Build history of the part. All positions in model axes, mm. A direction names the side the tool comes from. Give positions to 0.01 mm unless a question says otherwise; leave off trailing zeros. Write each loop counter-clockwise with the first axis right and the second up, starting at its lowest first coordinate (ties: lowest second). Pieces come first, ordered by that corner, then holes. Notation, with made-up numbers: M -34.5,-17.75 L -2.5,-17.75 A26 cw -2.5,4.25 Z; hole C -5.75,8 d10. An arc over 180 degrees is marked long. Return JSON: item names as keys, results as strings. Group by question number.
Q1. Wall check: probe 1 along Y at (x, z) = (-55, 27); probe 2 along Y at (x, z) = (-36.71, 14.75) (3 decimals); probe 3 along Y at (x, z) = (-51, 4). Give the ranges that are in metal, low to high.
Q2. Flat gauge pins, fed straight in: pin 1 Ø16 at (x, y) = (-55, 55) entering from -Z; pin 2 Ø10 at (x, y) = (36.71, -52.425) entering from +Z; pin 3 Ø9.5 at (x, y) = (53, -59.5) entering from -Z. Where does each tip first touch, or does it go through?
Q3. Tool access for faces 1 (the cylindrical face through (-48.371, 37.987, 12.422)), 2 (the cylindrical face through (16.128, -25.296, 33.997)): list every direction of +Z, -Z, +X, -X, +Y, -Y with a clear straight run to the whole face (end or side of a thin tool).
Q4. Pull direction Y, two halves, no side cores. Call faces 3 (the cylindrical face through (45.939, 57.854, 19.72)), 4 (the flat face through (-1, -67, 33)), 5 (the flat face through (-60, 1, 67)): +Y half, -Y half, draft (parallel to the pull), parting line (faces both ways), or undercut.
Q5. Band-saw the part on C-C, the plane z = 54. Give the cut face in (x, y), then the cut area to 3 significant figures.
Q6. Band-saw the part on A-A, the plane y = 0. Give the cut face in (x, z), then the cut area to 3 significant figures.
Q7. Band-saw the part on D-D, the plane z = 21.5. Count the separate pieces of the cut face and the enclosed holes in it, then the cut area to 3 significant figures.
from build123d import *

# Parameters (mm, degrees)
SKETCH1_W                  = 134
SKETCH1_H                  = 134
BOSS_EXTRUDE1_DEPTH        = 67
FILLET1_R                  = 12
SKETCH2_R                  = 30
CUT_EXTRUDE1_DEPTH         = 67
BOSS_EXTRUDE2_START        = 2
SKETCH3_R                  = 58
SKETCH3_R_2                = 30
BOSS_EXTRUDE2_DEPTH        = 2
SKETCH4_R                  = 58
SKETCH4_R_2                = 30
BOSS_EXTRUDE3_DEPTH        = 2
SKETCH5_R                  = 7
CUT_EXTRUDE2_DEPTH         = 160
SKETCH6_R                  = 9.5
CUT_EXTRUDE3_DEPTH         = 40
SIZE_MM_DOWEL_HOLE_1_D     = 8.5
SIZE_MM_DOWEL_HOLE_1_DEPTH = 24.5
SIZE_MM_DOWEL_HOLE_1_TIP   = 2.553657631
SIZE_MM_DOWEL_HOLE_2_D     = 8.5
SIZE_MM_DOWEL_HOLE_2_DEPTH = 24.5
SIZE_MM_DOWEL_HOLE_2_TIP   = 2.553657631
SIZE_MM_DOWEL_HOLE_3_D     = 8.6
SIZE_MM_DOWEL_HOLE_3_DEPTH = 10
SIZE_MM_DOWEL_HOLE_3_TIP   = 2.583700662


with BuildPart() as part:
    # Sketch1 → Boss-Extrude1 (new body)
    with BuildSketch(Plane.XY):
        Rectangle(SKETCH1_W, SKETCH1_H)
    extrude(amount=BOSS_EXTRUDE1_DEPTH)

    # Fillet1
    fillet1_edges = [part.edges().sort_by_distance(p)[0] for p in [
        (-67, 67, 33.5),
        (67, 67, 33.5),
        (67, -67, 33.5),
        (-67, -67, 33.5),
    ]]
    fillet(fillet1_edges, radius=FILLET1_R)

    # Sketch2 → Cut-Extrude1 (cut)
    with BuildSketch(Plane.XY.offset(67)):
        Circle(SKETCH2_R)
    extrude(amount=-CUT_EXTRUDE1_DEPTH, mode=Mode.SUBTRACT)

    # Sketch3 → Boss-Extrude2 (add)
    with BuildSketch(Plane.XY.offset(67).offset(BOSS_EXTRUDE2_START)):
        Circle(SKETCH3_R)
        Circle(SKETCH3_R_2, mode=Mode.SUBTRACT)
    extrude(amount=-BOSS_EXTRUDE2_DEPTH)

    # Sketch4 → Boss-Extrude3 (add)
    with BuildSketch(Plane(origin=(0, 0, 0), x_dir=(-1, 0, 0), z_dir=(0, 0, -1))):
        with Locations(Location((0, 0, 0), (0, 0, 180))):
            Circle(SKETCH4_R)
        with Locations(Location((0, 0, 0), (0, 0, 180))):
            Circle(SKETCH4_R_2, mode=Mode.SUBTRACT)
    extrude(amount=BOSS_EXTRUDE3_DEPTH)

    # Sketch5 → Cut-Extrude2 (cut)
    with BuildSketch(Plane(origin=(0, 0, 0), x_dir=(-1, 0, 0), z_dir=(0, 0, -1))):
        with Locations((-55, 55)):
            Circle(SKETCH5_R)
        with Locations((55, 55)):
            Circle(SKETCH5_R)
        with Locations((55, -55)):
            Circle(SKETCH5_R)
        with Locations((-55, -55)):
            Circle(SKETCH5_R)
    extrude(amount=-CUT_EXTRUDE2_DEPTH, mode=Mode.SUBTRACT)

    # Sketch6 → Cut-Extrude3 (cut)
    with BuildSketch(Plane(origin=(0, 0, 0), x_dir=(-1, 0, 0), z_dir=(0, 0, -1))):
        with Locations((-55, 55)):
            Circle(SKETCH6_R)
        with Locations((55, 55)):
            Circle(SKETCH6_R)
        with Locations((55, -55)):
            Circle(SKETCH6_R)
        with Locations((-55, -55)):
            Circle(SKETCH6_R)
    extrude(amount=-CUT_EXTRUDE3_DEPTH, mode=Mode.SUBTRACT)

    # Size mm Dowel hole 1
    with Locations(Plane(origin=(0, 0, 0), x_dir=(-1, 0, 0), z_dir=(0, 0, -1))):
        with Locations((-36.71, 52.425), (36.71, 52.425), (36.71, -52.425), (-36.71, -52.425)):
            Hole(SIZE_MM_DOWEL_HOLE_1_D / 2, depth=SIZE_MM_DOWEL_HOLE_1_DEPTH)
            with Locations((0, 0, -(SIZE_MM_DOWEL_HOLE_1_DEPTH + SIZE_MM_DOWEL_HOLE_1_TIP / 2))):  # 118° drill point
                Cone(0, SIZE_MM_DOWEL_HOLE_1_D / 2, SIZE_MM_DOWEL_HOLE_1_TIP, mode=Mode.SUBTRACT)

    # Size mm Dowel hole 2
    with Locations(Plane(origin=(0, 0, 0), x_dir=(-1, 0, 0), z_dir=(0, 0, -1))):
        with Locations((-52.425, 36.71), (52.425, 36.71), (52.425, -36.71), (-52.425, -36.71)):
            Hole(SIZE_MM_DOWEL_HOLE_2_D / 2, depth=SIZE_MM_DOWEL_HOLE_2_DEPTH)
            with Locations((0, 0, -(SIZE_MM_DOWEL_HOLE_2_DEPTH + SIZE_MM_DOWEL_HOLE_2_TIP / 2))):  # 118° drill point
                Cone(0, SIZE_MM_DOWEL_HOLE_2_D / 2, SIZE_MM_DOWEL_HOLE_2_TIP, mode=Mode.SUBTRACT)

    # Size mm Dowel hole 3
    with Locations(Plane(origin=(0, 67, 0), x_dir=(1, 0, 0), z_dir=(0, 1, 0))):
        with Locations((-20, -15), (20, -15)):
            Hole(SIZE_MM_DOWEL_HOLE_3_D / 2, depth=SIZE_MM_DOWEL_HOLE_3_DEPTH)
            with Locations((0, 0, -(SIZE_MM_DOWEL_HOLE_3_DEPTH + SIZE_MM_DOWEL_HOLE_3_TIP / 2))):  # 118° drill point
                Cone(0, SIZE_MM_DOWEL_HOLE_3_D / 2, SIZE_MM_DOWEL_HOLE_3_TIP, mode=Mode.SUBTRACT)


solid = part.part
From the geometry:
{
 "1": {"probe 1": "y = -67 to -64.5, -45.5 to 45.5, 64.5 to 67", "probe 2": "y = -67 to -56.675, -48.175 to 48.175, 56.675 to 67", "probe 3": "y = -67 to -63.62, -46.38 to -40.71, -32.71 to 32.71, 40.71 to 46.38, 63.62 to 67"},
 "2": {"pin 1": "stops at z = 40", "pin 2": "stops at z = 67", "pin 3": "stops at z = 0"},
 "3": {"face 1": "-Z", "face 2": "+Z, -Z"},
 "4": {"face 3": "undercut", "face 4": "-Y half", "face 5": "draft"},
 "5": {"outline": "M -67,-55 A12 ccw -55,-67 L 55,-67 A12 ccw 67,-55 L 67,55 A12 ccw 55,67 L -55,67 A12 ccw -67,55 Z; hole C -55,-55 d14; hole C -55,55 d14; hole C 0,0 d60; hole C 55,-55 d14; hole C 55,55 d14", "area": "14,400 mm^2"},
 "6": {"outline": "M -67,0 L -58,0 L -58,-2 L -30,-2 L -30,69 L -58,69 L -58,67 L -67,67 Z; M 30,-2 L 58,-2 L 58,0 L 67,0 L 67,67 L 58,67 L 58,69 L 30,69 Z", "area": "5,180 mm^2"},
 "7": {"separate pieces": "1", "enclosed holes": "13", "area": "13,400 mm^2"}
}
